```python
from build123d import *

# Parameters (mm, degrees)
BOSS_EXTRUDE1_DEPTH = 195
CHAMFER1_SIZE       = 30
CHAMFER1_SIZE2      = 5.289809421
FILLET1_R           = 2


with BuildPart() as part:
    # Sketch1 → Boss-Extrude1 (new, symmetric)
    with BuildSketch(Plane.XY):
        Polygon((0, -5.5), (0, 5.5), (-6, 5.5), (-6, 3.3), (-14, 3.3), (-14, -3.3), (-6, -3.3), (-6, -5.5), align=None)
    extrude(amount=BOSS_EXTRUDE1_DEPTH, both=True)

    # Chamfer1
    chamfer1_edges = [part.edges().sort_by_distance(p)[0] for p in [
        (-14, 0, 195),
        (-14, 0, -195),
    ]]
    chamfer1_side = [part.faces().sort_by_distance(p)[0] for p in [
        (-14, 0, 0),
    ]]
    chamfer(chamfer1_edges, length=CHAMFER1_SIZE, length2=CHAMFER1_SIZE2, reference=chamfer1_side[0])

    # Fillet1
    fillet1_edges = [part.edges().sort_by_distance(p)[0] for p in [
        (-14, 0, 165),
        (-14, 0, -165),
        (-8.710190579, 0, -195),
        (-8.710190579, 0, 195),
    ]]
    fillet(fillet1_edges, radius=FILLET1_R)


solid = part.part
```
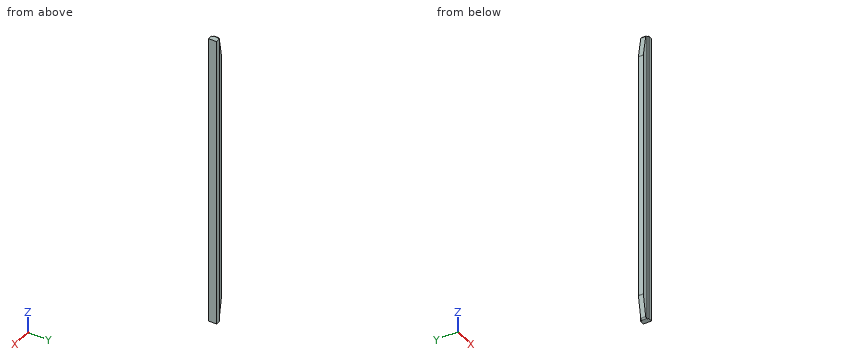
CAD build for the part. Positions are in the model's coordinates, mm. Coordinates: 2 decimals unless noted, no trailing zeros. Order: outer loops, then holes, each group sorted by start corner. A loop starts at its lowest first (then second) coordinate and runs counter-clockwise, first axis right, second up.
(1) Pin check, flat tips, straight feed: pin 1 Ø2 at (x, z) = (-12, 131.5) entering from -Y; pin 2 Ø2.5 at (x, z) = (-11.5, 73.5) entering from +Y. Stop position of each tip, or through.
Solution:
pin 1: stops at y = -3.3
pin 2: stops at y = 3.3
(2) Drill centre lines: L1, parallel to X at y = 4.5, z = -26; L2, parallel to Y at x = -13, z = -40; L3, parallel to Z at x = -7.25, y = -1.5. Where is each one in solid material? Low to high.
Solution:
L1: x = -6 to 0
L2: y = -3.3 to 3.3
L3: z = -194.99 to 194.99
(3) Saw through at A-A, the plane y = -1. Write the cut outline in (x, z), and give its area (3 significant figures).
Solution:
outline: (-14, -164.83) arc R2 ccw to (-13.97, -165.17) - (-9, -193.35) arc R2 ccw to (-7.03, -195) - (0, -195) - (0, 195) - (-7.03, 195) arc R2 ccw to (-9, 193.35) - (-13.97, 165.17) arc R2 ccw to (-14, 164.83) - close
area: 5,300 mm2
(4) Saw through at B-B, the plane z = 104.5. Write the cut outline in (x, y).
Solution:
outline: (-14, -3.3) - (-6, -3.3) - (-6, -5.5) - (0, -5.5) - (0, 5.5) - (-6, 5.5) - (-6, 3.3) - (-14, 3.3) - close
